For this review, use the dimensioned drawing (mm, ordinates from the lowest corner) and the shaded views. Round coordinates to 2 decimals unless told otherwise and drop trailing zeros. Write each loop counter-clockwise with the first axis right and the second up, starting at its lowest first coordinate (ties: lowest second). Pieces come first, ordered by that corner, then holes. Notation, with made-up numbers: M 39.5,-18.75 L 78.5,-18.75 A9 ccw 78.5,-9.75 Z; hole C 25,19 d9. An arc over 180 degrees is marked long. One line per question, with ' | ' between items. Start each with the question number.
Item 1: For L1, parallel to X at y = 302, z = 3.25; L2, parallel to Y at x = 15, z = 12.25; L3, parallel to Y at x = 11, z = 6.75, list the stretches that pass through material, from the lowest coordinate up.
Item 2: Add section A-A, the plane y = 302. State the section outline as (x, z) points.
Item 3: Insertion check: pin 1 Ø7.5 at (x, y) = (15, 302) entering from -Z. The pin has a flat end and moves straight along its axis. Give the tip position at first contact, or say it passes through.
Item 4: Add section B-B, the plane x = 15. Give the number of separate pieces and of enclosed holes in the cut face, and give its area (3 significant figures).
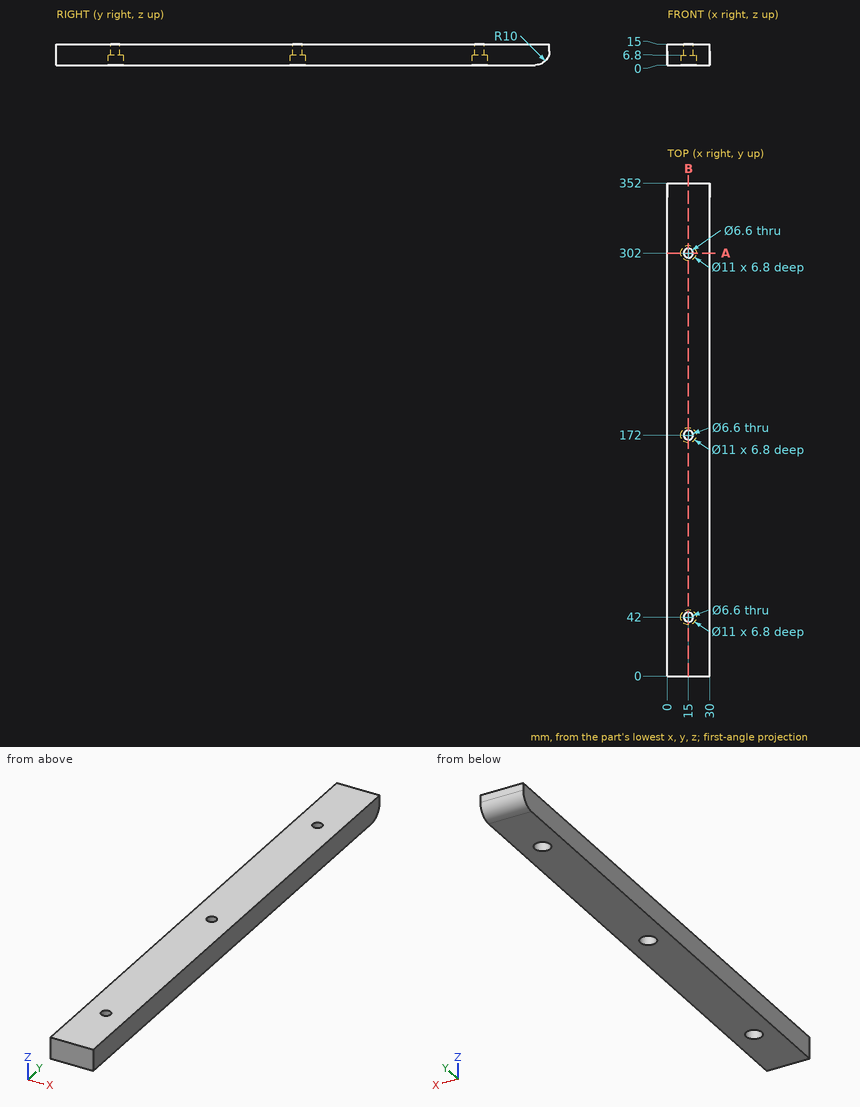
Computed values:
1) L1: x = 0 to 9.5, 20.5 to 30 | L2: y = 0 to 38.7, 45.3 to 168.7, 175.3 to 298.7, 305.3 to 352 | L3: y = 0 to 38.23, 45.77 to 168.23, 175.77 to 298.23, 305.77 to 351.46
2) outline: M 0,0 L 9.5,0 L 9.5,6.8 L 11.7,6.8 L 11.7,15 L 0,15 Z; M 18.3,6.8 L 20.5,6.8 L 20.5,0 L 30,0 L 30,15 L 18.3,15 Z
3) pin 1: stops at z = 6.8
4) separate pieces: 4 | enclosed holes: 0 | area: 4,870 mm^2
